Could you check a few things on this drawing? It's one solid part, dimensions in mm from its lowest x, y, z. A direction names the side the tool comes from. Give positions to 0.01 mm unless a question says otherwise; leave off trailing zeros. Order: outer loops, then holes, each group sorted by start corner. A loop starts at its lowest first (then second) coordinate and runs counter-clockwise, first axis right, second up. Notation, with made-up numbers: M 10,21 L 34,21 A28 ccw 34,43 Z; hole C 13.25,16.5 d6. An arc over 180 degrees is marked long. Return JSON: item names as keys, results as strings. Group by question number.
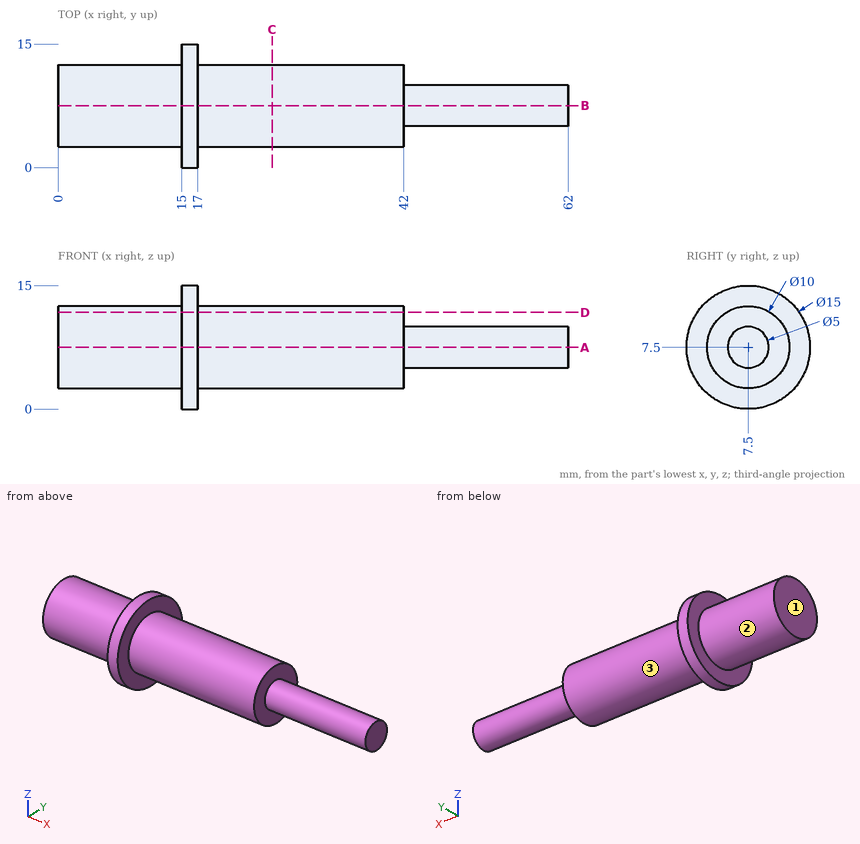
1. Imagine slicing it at C-C, the plane x = 26. Please give me the cut outline in (y, z).
2. Which directions (+Z, -Z, +X, -X, +Y, -Y) give clear straight access to the entire face, cutting with the end or side of a thin tool? Please do the marked faces 1, 2 and 3.
3. Imagine slicing it at D-D, the plane z = 11.75. Please give me the cut outline in (x, y), plus the area to 3 significant figures.
4. Imagine slicing it at A-A, the plane z = 7.5. Please give me the cut outline in (x, y).
5. I need wall thicknesses on L1, parallel to X at y = 11.75, z = 8.75; L2, parallel to Y at x = 45.5, z = 7.25; L3, parallel to X at y = 13, z = 5. Which ranges of each line are inside material? Lowest first, please. Write a range as from..to.
6. For pin 1 (5 mm diameter, centred on x = 6.5, y = 8, fed in from +Z); pin 2 (8 mm diameter, centred on x = 39, z = 9, fed in from -Y); pin 3 (5 mm diameter, centred on x = 37, z = 3.5, fed in from +Y), each with a flat end and sliding along its axis, tell me the tip position at first contact or that it passes through.
Values:
{
 "1": {"outline": "C 7.5,7.5 d10"},
 "2": {"face 1": "+Z, -Z, -X, +Y, -Y", "face 2": "-X", "face 3": "+X"},
 "3": {"outline": "M 0,4.87 L 15,4.87 L 15,1.32 L 17,1.32 L 17,4.87 L 42,4.87 L 42,10.13 L 17,10.13 L 17,13.68 L 15,13.68 L 15,10.13 L 0,10.13 Z", "area": "235 mm²"},
 "4": {"outline": "M 0,2.5 L 15,2.5 L 15,0 L 17,0 L 17,2.5 L 42,2.5 L 42,5 L 62,5 L 62,10 L 42,10 L 42,12.5 L 17,12.5 L 17,15 L 15,15 L 15,12.5 L 0,12.5 Z"},
 "5": {"L1": "x = 0..42", "L2": "y = 5.01..9.99", "L3": "x = 15..17"},
 "6": {"pin 1": "stops at z = 12.5", "pin 2": "stops at y = 2.5", "pin 3": "stops at y = 12.27"}
}
